Build history of the part. All positions in model axes, mm. A direction names the side the tool comes from. Coordinates: 2 decimals unless noted, no trailing zeros. Write each loop counter-clockwise with the first axis right and the second up, starting at its lowest first coordinate (ties: lowest second). Pieces come first, ordered by that corner, then holes.
```python
from build123d import *

# Parameters (mm, degrees)
BOSS_EXTRUDE_1_DEPTH     = 503.38
CUT_EXTRUDE_1_DEPTH      = 506.410154627
CUT_EXTRUDE_1_DEPTH_BACK = 506.410154627


with BuildPart() as part:
    # Sketch 1 → Boss-Extrude 1 (new, symmetric)
    with BuildSketch(Plane.XY):
        with BuildLine():
            Line((0, 32), (-24, 32))
            ThreePointArc((-24, 32), (-29.656854249, 29.656854249), (-32, 24))
            Line((-32, 24), (-32, 0))
            Line((-32, 0), (-32, -24))
            ThreePointArc((-32, -24), (-29.656854249, -29.656854249), (-24, -32))
            Line((-24, -32), (24, -32))
            ThreePointArc((24, -32), (29.656854249, -29.656854249), (32, -24))
            Line((32, -24), (32, 0))
            Line((32, 0), (32, 24))
            ThreePointArc((32, 24), (29.656854249, 29.656854249), (24, 32))
            Line((24, 32), (0, 32))
        make_face()
        with BuildLine():
            Line((0, 28), (-24, 28))
            ThreePointArc((-24, 28), (-26.828427125, 26.828427125), (-28, 24))
            Line((-28, 24), (-28, 0))
            Line((-28, 0), (-28, -24))
            ThreePointArc((-28, -24), (-26.828427125, -26.828427125), (-24, -28))
            Line((-24, -28), (24, -28))
            ThreePointArc((24, -28), (26.828427125, -26.828427125), (28, -24))
            Line((28, -24), (28, 0))
            Line((28, 0), (28, 24))
            ThreePointArc((28, 24), (26.828427125, 26.828427125), (24, 28))
            Line((24, 28), (0, 28))
        make_face(mode=Mode.SUBTRACT)
    extrude(amount=BOSS_EXTRUDE_1_DEPTH, both=True)

    # Sketch 2 → Cut-Extrude 1 (cut, two sides: drawn at the far end of the back side and taken through both)
    with BuildSketch(Plane(origin=(0, 0, 0), x_dir=(0, 0, -1), z_dir=(1, 0, 0)).offset(-CUT_EXTRUDE_1_DEPTH_BACK)):
        Polygon((-503.38, 32), (-439.38, -32), (-503.38, -32), align=None)
        Polygon((503.38, -32), (503.38, 32), (439.38, -32), align=None)
    extrude(amount=CUT_EXTRUDE_1_DEPTH + CUT_EXTRUDE_1_DEPTH_BACK, mode=Mode.SUBTRACT)


solid = part.part
```
1. Probe line 1 along Y through (x, z) = (3, -225); line 2 along X through (y, z) = (26.5, 47.5). List the from-to ranges inside material, lowest first.
Computed values:
line 1: y = -32 to -28, 28 to 32
line 2: x = -31.6 to -27.12, 27.12 to 31.6
2. Saw through at C-C on z = 208.5. List the corners of the cut face in (x, y), plus the area to 3 significant figures.
Computed values:
outline: (-32, -24) arc R8 ccw to (-24, -32) - (24, -32) arc R8 ccw to (32, -24) - (32, 24) arc R8 ccw to (24, 32) - (-24, 32) arc R8 ccw to (-32, 24) - close; hole (-28, -24) arc R4 ccw to (-24, -28) - (24, -28) arc R4 ccw to (28, -24) - (28, 24) arc R4 ccw to (24, 28) - (-24, 28) arc R4 ccw to (-28, 24) - close
area: 919 mm2
3. Saw through at A-A on y = -9.5. List the corners of the cut face in (x, z).
Computed values:
outline: (-32, -461.88) - (-28, -461.88) - (-28, 461.88) - (-32, 461.88) - close; (28, -461.88) - (32, -461.88) - (32, 461.88) - (28, 461.88) - close
4. Mould opens along Y. For faces 1 (the face through (0, -32, 6)), 2 (the face through (-32, 0, 7)), 3 (the face through (-28, 0, 7)) say: +Y half, -Y half, draft (parallel to the pull), parting line (faces both ways), or undercut.
Computed values:
face 1: -Y half
face 2: draft
face 3: undercut
5. 3-axis set-ups, long thin cutter, end or side, ignore diameter. For faces 4 (the face through (0, 32, 7)), 5 (the face through (0, 28, 7)): which of +Z, -Z, +X, -X, +Y, -Y reach the whole face in a straight line?
Computed values:
face 4: +Z, -Z, +X, -X, +Y
face 5: +Z, -Z
6. Saw through at B-B on x = 15. List the corners of the cut face in (y, z).
Computed values:
outline: (-32, -439.38) - (-28, -443.38) - (-28, 443.38) - (-32, 439.38) - close; (28, -499.38) - (32, -503.38) - (32, 503.38) - (28, 499.38) - close
